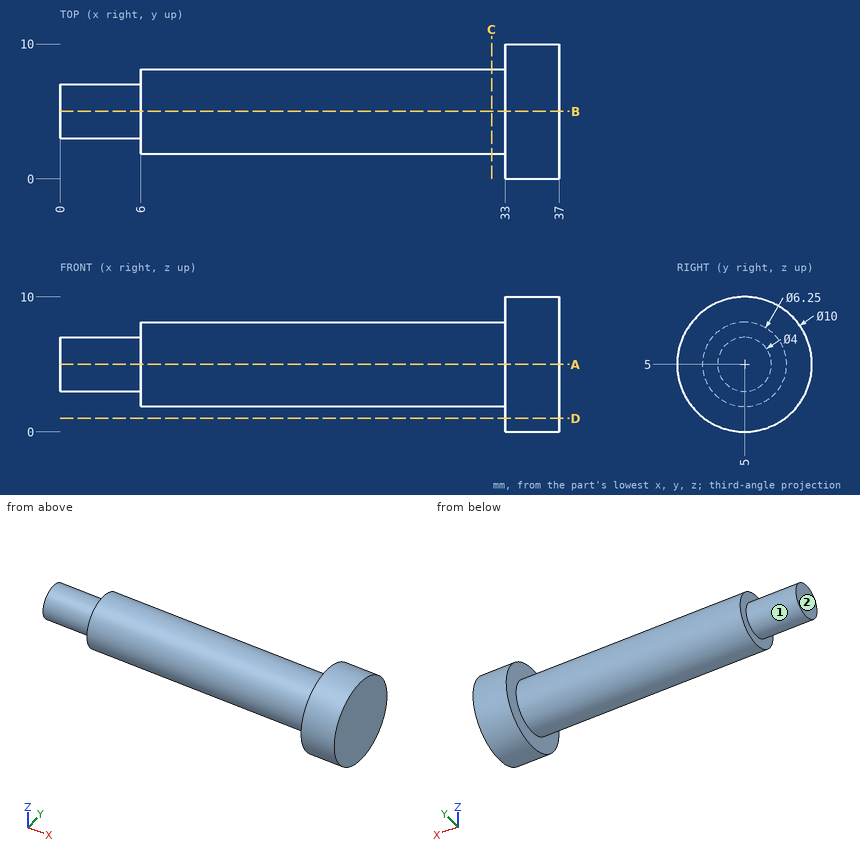
Input: dimensioned drawing with shaded views. Units: mm. Origin: part minimum x, y, z. A direction names the side the tool comes from. Give positions to 0.01 mm unless a question says otherwise; leave off trailing zeros. Loops run counter-clockwise (first coordinate to the right, second up) from the corner with the lowest first, then second, coordinate; pieces in that order, holes last. Notation, with made-up numbers: (86.5, 3) -> (132.5, 3) arc R13 cw to (132.5, 9) -> close; hole circle Ø10 at (5, -6.75). An arc over 180 degrees is marked (long way). Return JSON: item names as keys, results as strings.
Item 1: Section A-A, the plane z = 5. Output: boundary loops of the cut face in (x, y) (3 decimals).
Filled in:
{"outline": "(0, 3) -> (6, 3) -> (6, 1.875) -> (33, 1.875) -> (33, 0) -> (37, 0) -> (37, 10) -> (33, 10) -> (33, 8.125) -> (6, 8.125) -> (6, 7) -> (0, 7) -> close"}
Item 2: Line query: line 1 (X direction, y = 9.25, z = 4.5); line 2 (X direction, y = 5, z = 8); line 3 (Y direction, x = 24.5, z = 7). Output: solid intervals per line, ascending.
Filled in:
{"line 1": "33 to 37", "line 2": "6 to 37", "line 3": "2.6 to 7.4"}
Item 3: Pin query (flat end, axial travel): P1, Ø5, axis at x = 11, y = 3.5, coming from the -Z side (3 decimals); P2, Ø1.5, axis at x = 15.5, y = 8, coming from the -Z side; P3, Ø5, axis at y = 3.5, z = 4.5, coming from the -X side. Return the tip coordinate at first contact, or that it passes through.
Filled in:
{"P1": "z = 1.875", "P2": "z = 2.83", "P3": "x = 0"}
Item 4: Section D-D, the plane z = 1. Output: boundary loops of the cut face in (x, y).
Filled in:
{"outline": "(33, 2) -> (37, 2) -> (37, 8) -> (33, 8) -> close"}
Item 5: Section C-C, the plane x = 32. Output: boundary loops of the cut face in (y, z) (3 decimals).
Filled in:
{"outline": "circle Ø6.25 at (5, 5)"}
Item 6: Access query for the marked faces 1 and 2. Directions: +Z, -Z, +X, -X, +Y, -Y. A direction counts if a zero-diameter tool reaches every point of the face in a straight line with its end or side. Return the directions, or none.
Filled in:
{"face 1": "-X", "face 2": "+Z, -Z, -X, +Y, -Y"}
